```python
from build123d import *

# Parameters (mm, degrees)
CHAMFER_1_SIZE = 1


with BuildPart() as part:
    # 草图1 → 旋转1 (revolve)
    with BuildSketch(Plane.XY, mode=Mode.PRIVATE) as revolve_1_sk:
        Polygon((-116.444838016, -84.118352239), (-122.444838016, -84.118352239), (-122.444838016, -85.118352239), (-124.444838016, -85.118352239), (-124.444838016, -82.868352239), (-129.444838016, -82.868352239), (-129.444838016, -81.118352239), (-134.444838016, -81.118352239), (-134.444838016, -89.118352239), (-116.444838016, -89.118352239), align=None)
    revolve(revolve_1_sk.sketch.rotate(Axis((-129.444838016, -89.118352239, 0), (1, 0, 0)), 90), axis=Axis((-129.444838016, -89.118352239, 0), (1, 0, 0)))

    # 倒角1
    chamfer_1_edges = [part.edges().sort_by_distance(p)[0] for p in [
        (-124.444838016, -89.118352239, -6.25),
        (-134.444838016, -89.118352239, -8),
        (-129.444838016, -89.118352239, -8),
    ]]
    chamfer(chamfer_1_edges, length=CHAMFER_1_SIZE)


solid = part.part
```
Source: CAD feature listing. Evaluate the final solid. Frame: model axes, mm. A direction names the side the tool comes from. Give positions to 0.01 mm unless a question says otherwise; leave off trailing zeros. Write each loop counter-clockwise with the first axis right and the second up, starting at its lowest first coordinate (ties: lowest second). Pieces come first, ordered by that corner, then holes.
1. Section query A-A (z = 0). Return the cut outline in (x, y), then the cut area to 4 significant figures.
2. First-contact query: pin 1 (2 mm diameter, centred on x = -132, y = -95.5, fed in from -Z); pin 2 (5 mm diameter, centred on x = -124, y = -84, fed in from -Z); pin 3 (2 mm diameter, centred on y = -92.5, z = 5.5, fed in from +X). Flat tips, straight axial feed; report the tip coordinate or a pass-through.
3. Section query B-B (x = -126.25). Return the cut outline in (y, z), then the cut area to 3 significant figures.
4. Pull-direction query (X, two-part tool) for faces 1 (the face through (-116.445, -89, 0)), 2 (the face through (-127.473, -95.315, -0.814)), 3 (the face through (-122.445, -88, -4)); classes: +X half, -X half, draft (parallel to the pull), parting line (faces both ways), or undercut.
5. Section query C-C (x = -131). Return the cut outline in (y, z).
6. Material intervals for line 1 along Z through (x, y) = (-126.75, -89.25); line 2 along X through (y, z) = (-84.75, -0.5); line 3 along Z through (x, y) = (-117, -89.25), sorted ascending.
7. Access query for faces 4 (the face through (-119.487, -93.334, 2.688)), 5 (the face through (-123.46, -85.57, 1.85)), 6 (the face through (-132, -81.3, -1.7)). Directions: +Z, -Z, +X, -X, +Y, -Y. A direction counts if a zero-diameter tool reaches every point of the face in a straight line with its end or side. Return the directions, or none.
Output values:
1. outline: (-134.44, -96.12) - (-133.44, -97.12) - (-130.44, -97.12) - (-129.44, -96.12) - (-129.44, -95.37) - (-125.44, -95.37) - (-124.44, -94.37) - (-124.44, -93.12) - (-122.44, -93.12) - (-122.44, -94.12) - (-116.44, -94.12) - (-116.44, -84.12) - (-122.44, -84.12) - (-122.44, -85.12) - (-124.44, -85.12) - (-124.44, -83.87) - (-125.44, -82.87) - (-129.44, -82.87) - (-129.44, -82.12) - (-130.44, -81.12) - (-133.44, -81.12) - (-134.44, -82.12) - close
1. area: 215.5 mm2
2. pin 1: stops at z = -5.92
2. pin 2: stops at z = -5.44
2. pin 3: stops at x = -124.65
3. outline: circle Ø12.5 at (-89.12, 0)
3. area: 123 mm2
4. face 1: +X half
4. face 2: draft
4. face 3: undercut
5. outline: circle Ø16 at (-89.12, 0)
6. line 1: z = -6.25 to 6.25
6. line 2: x = -134.44 to -124.44, -122.44 to -116.44
6. line 3: z = -5 to 5
7. face 4: +X
7. face 5: none
7. face 6: +X, -X
